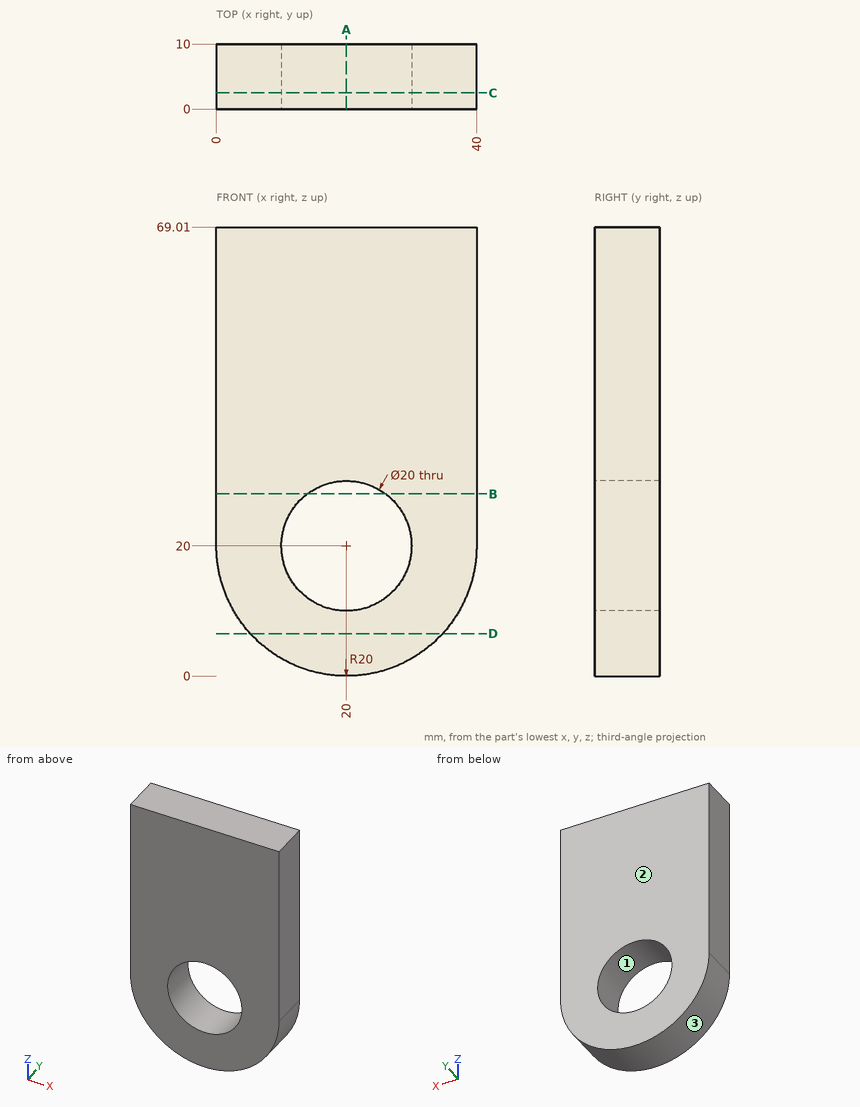
Drawing for the job (mm, zero at the part's lowest x, y, z). Round coordinates to 2 decimals unless told otherwise and drop trailing zeros. Order: outer loops, then holes, each group sorted by start corner. A loop starts at its lowest first (then second) coordinate and runs counter-clockwise, first axis right, second up. Notation, with made-up numbers: (85.25, 19) -> (98.25, 19) arc R26 cw to (98.25, 48) -> close; hole circle Ø1 at (-32, -1.75). An arc over 180 degrees is marked (long way). Put each result on its own line as item: value.
Q1. Band-saw the part on A-A (x = 20). Give the cut face in (y, z), and give its area (3 significant figures).
From the geometry:
outline: (0, 0) -> (10, 0) -> (10, 10) -> (0, 10) -> close; (0, 30) -> (10, 30) -> (10, 69.01) -> (0, 69.01) -> close
area: 490 mm2
Q2. Band-saw the part on B-B (z = 28). Give the cut face in (x, y).
From the geometry:
outline: (0, 0) -> (14, 0) -> (14, 10) -> (0, 10) -> close; (26, 0) -> (40, 0) -> (40, 10) -> (26, 10) -> close
Q3. Pin check, flat tips, straight feed: pin 1 Ø12 at (x, z) = (21.5, 20.5) entering from +Y; pin 2 Ø1.5 at (x, y) = (15.5, 5) entering from -Z. Stop position of each tip, or through.
From the geometry:
pin 1: passes through
pin 2: stops at z = 0.35
Q4. Pull direction Z, two halves, no side cores. Call the marked faces 1, 2 and 3: pulls with the +Z half, pulls with the -Z half, needs draft (parallel to the pull), parting line crosses it, or undercut.
From the geometry:
face 1: undercut
face 2: needs draft
face 3: pulls with the -Z half
Q5. Band-saw the part on C-C (y = 2.5). Give the cut face in (x, z), and give its area (3 significant figures).
From the geometry:
outline: (0, 20) arc R20 ccw to (40, 20) -> (40, 69.01) -> (0, 69.01) -> close; hole circle Ø20 at (20, 20)
area: 2,270 mm2
Q6. Wall check: line 1 (Z direction, x = 20.5, y = 4); line 2 (Z direction, x = 14.5, y = 4.5); line 3 (X direction, y = 9.75, z = 15.5). Give the ranges that are in metal, low to high. Write a range as [from, to].
From the geometry:
line 1: z = [0.01, 10.01], [29.99, 69.01]
line 2: z = [0.77, 11.65], [28.35, 69.01]
line 3: x = [0.51, 11.07], [28.93, 39.49]
Q7. Band-saw the part on D-D (z = 6.5). Give the cut face in (x, y).
From the geometry:
outline: (5.24, 0) -> (34.76, 0) -> (34.76, 10) -> (5.24, 10) -> close
